Could you check a few things on this model? Use its own coordinates, in mm. Face numbers are marked on the shaded views. A direction names the side the tool comes from. Give positions to 0.01 mm unless a question says otherwise; leave off trailing zeros. Write each loop counter-clockwise with the first axis right and the second up, starting at its lowest first coordinate (ties: lowest second). Pieces come first, ordered by that corner, then holes. Notation, with made-up numbers: (-34.75, -34.5) - (-18.75, -34.5) arc R12 cw to (-18.75, -16.5) - close; hole circle Ø4 at (-10, 45.5). An arc over 180 degrees is marked (long way). Answer as a JSON object with one key per item and string values. Group by question number.
```python
from build123d import *

# Parameters (mm, degrees)
SKETCH_1_W      = 116
SKETCH_1_H      = 116
EXTRUDE_1_DEPTH = 3
SKETCH_2_W      = 91
SKETCH_2_H      = 91
EXTRUDE_2_DEPTH = 17


with BuildPart() as part:
    # 草图1 → 凸台-拉伸1 (new body)
    with BuildSketch(Plane.XY):
        Rectangle(SKETCH_1_W, SKETCH_1_H)
    extrude(amount=EXTRUDE_1_DEPTH)

    # 草图2 → 凸台-拉伸2 (add)
    with BuildSketch(Plane.XY.offset(3)):
        Rectangle(SKETCH_2_W, SKETCH_2_H)
    extrude(amount=EXTRUDE_2_DEPTH)


solid = part.part
```
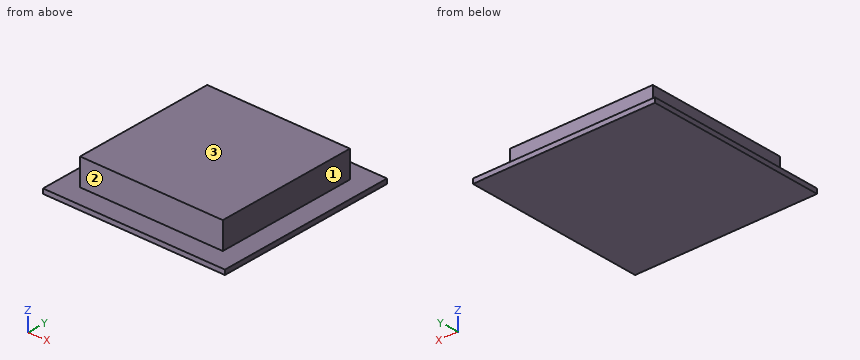
(1) For the marked faces 1, 2 and 3, which set-ups out of +Z, -Z, +X, -X, +Y, -Y let a thin tool reach every point of the face, with its end or its side?
(2) I want a section at C-C, the plane z = 9.25. Please give me the cut outline in (x, y).
(3) I want a section at A-A, the plane x = 24.5. Please give me the cut outline in (y, z).
(4) I need wall thicknesses on L1, parallel to X at y = -9, z = 5.25; L2, parallel to Z at x = 46.5, y = -8. Which ranges of each line are inside material? Lowest first, please.
(5) I want a section at D-D, the plane x = -47.5. Please give me the cut outline in (y, z).
(6) Will these pins go through, and if not, where does the flat tip stop? P1, Ø4, axis at y = 23.5, z = 9.5, coming from the +X side; P2, Ø5, axis at x = -10, z = 11, coming from the +Y side; P3, Ø12, axis at x = -3, z = 12.5, coming from the -Y side.
Entries:
{
 "1": {"face 1": "+Z, +X, +Y, -Y", "face 2": "+Z, +X, -X, -Y", "face 3": "+Z, +X, -X, +Y, -Y"},
 "2": {"outline": "(-45.5, -45.5) - (45.5, -45.5) - (45.5, 45.5) - (-45.5, 45.5) - close"},
 "3": {"outline": "(-58, 0) - (58, 0) - (58, 3) - (45.5, 3) - (45.5, 20) - (-45.5, 20) - (-45.5, 3) - (-58, 3) - close"},
 "4": {"L1": "-45.5 to 45.5", "L2": "0 to 3"},
 "5": {"outline": "(-58, 0) - (58, 0) - (58, 3) - (-58, 3) - close"},
 "6": {"P1": "x = 45.5", "P2": "y = 45.5", "P3": "y = -45.5"}
}
